Input: part model. Units: mm. Frame: model coordinates. Face numbers are marked on the shaded views. A direction names the side the tool comes from. Round coordinates to 2 decimals unless told otherwise and drop trailing zeros. Order: outer loops, then holes, each group sorted by start corner. A loop starts at its lowest first (then second) coordinate and runs counter-clockwise, first axis right, second up. Notation, with made-up numbers: (24, 17) -> (66, 17) arc R13 ccw to (66, 22) -> close; hole circle Ø3 at (7.25, -18). An arc over 180 degrees is marked (long way). Use a Markdown table: item, result.
from build123d import *

# Parameters (mm, degrees)
BOSS_EXTRUDE_START   = 100
SKETCH_2_R           = 25
BOSS_EXTRUDE_1_DEPTH = 100
SKETCH_3_R           = 21
BOSS_EXTRUDE_2_DEPTH = 60


with BuildPart() as part:
    # Sketch 1 → Revolve 1 (revolve)
    with BuildSketch(Plane.XY, mode=Mode.PRIVATE) as revolve_1_sk:
        Polygon((-187.5, 0), (-187.5, 25), (-7.5, 25), (-7.5, 45), (7.5, 45), (7.5, 25), (187.5, 25), (187.5, 0), align=None)
    revolve(revolve_1_sk.sketch.rotate(Axis((-187.5, 0, 0), (1, 0, 0)), 180), axis=Axis((-187.5, 0, 0), (1, 0, 0)))

    # Sketch 2 → Boss-Extrude 1 (add)
    with BuildSketch(Plane(origin=(187.5, 0, 0), x_dir=(0, 0, -1), z_dir=(1, 0, 0)).offset(BOSS_EXTRUDE_START)):
        with Locations(Location((0, 0, 0), (0, 0, 270))):
            Circle(SKETCH_2_R)
    extrude(amount=-BOSS_EXTRUDE_1_DEPTH)

    # Sketch 3 → Boss-Extrude 2 (add)
    with BuildSketch(Plane.ZY.offset(187.5)):
        with Locations(Location((0, 0, 0), (0, 0, 270))):
            Circle(SKETCH_3_R)
    extrude(amount=BOSS_EXTRUDE_2_DEPTH)


solid = part.part
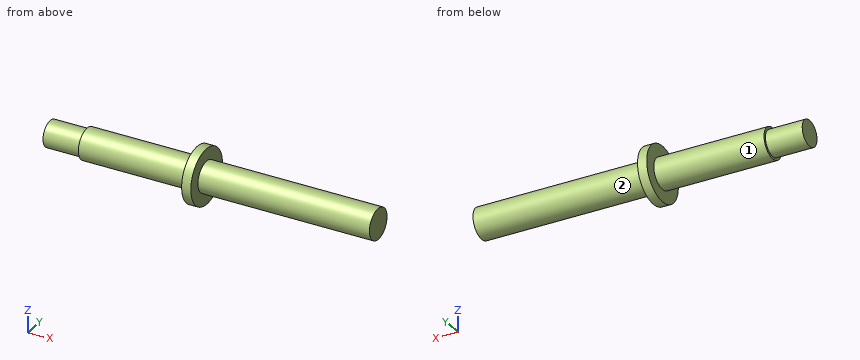
1) Cut plane A-A on z = 0. Return loops of the section in (x, y).
Answer key:
| item | result |
|---|---|
| outline | (-247.5, -21) -> (-187.5, -21) -> (-187.5, -25) -> (-7.5, -25) -> (-7.5, -45) -> (7.5, -45) -> (7.5, -25) -> (287.5, -25) -> (287.5, 25) -> (7.5, 25) -> (7.5, 45) -> (-7.5, 45) -> (-7.5, 25) -> (-187.5, 25) -> (-187.5, 21) -> (-247.5, 21) -> close |
2) Set-up query: the marked faces 1 and 2. Return all of +Z, -Z, +X, -X, +Y, -Y with unobstructed straight access to the full face (end or side cutting, diameter ignored); none if empty.
Answer key:
| item | result |
|---|---|
| face 1 | -X |
| face 2 | +X |
3) Cut plane C-C on x = -42. Return loops of the section in (y, z).
Answer key:
| item | result |
|---|---|
| outline | circle Ø50 at (0, 0) |
4) Cut plane D-D on z = -38. Return loops of the section in (x, y), and give its area (3 significant figures).
Answer key:
| item | result |
|---|---|
| outline | (-7.5, -24.1) -> (7.5, -24.1) -> (7.5, 24.1) -> (-7.5, 24.1) -> close |
| area | 723 mm^2 |
5) Ray query, probe 1 along X at (y, z) = (-21, 36.5); probe 2 along X at (y, z) = (-22, 6); probe 3 along Z at (x, y) = (-96, -0.5) (3 decimals). Return the intervals inside material, ascending.
Answer key:
| item | result |
|---|---|
| probe 1 | x = -7.5 to 7.5 |
| probe 2 | x = -187.5 to 287.5 |
| probe 3 | z = -24.995 to 24.995 |
6) Contact query for flat-ended pins moving along their axis: P1, Ø1, axis at x = -192, y = 1.5, coming from the +Z side; P2, Ø8, axis at x = 217.5, z = 27, coming from the -Y side; P3, Ø3, axis at y = -9, z = -32, coming from the +X side; P4, Ø8, axis at x = -127.5, y = 29.5, coming from the -Z side. Output: stop coordinate, or through.
Answer key:
| item | result |
|---|---|
| P1 | stops at z = 20.98 |
| P2 | stops at y = -9.8 |
| P3 | stops at x = 7.5 |
| P4 | passes through |
